```python
from build123d import *

# Parameters (mm, degrees)
SKETCH1_W           = 300
SKETCH1_H           = 80
BOSS_EXTRUDE1_DEPTH = 8
M8_TAPPED_HOLE1_D   = 6.8


with BuildPart() as part:
    # Sketch1 → Boss-Extrude1 (new body)
    with BuildSketch(Plane(origin=(0, 0, 0), x_dir=(1, 0, 0), z_dir=(0, 1, 0))):
        with Locations((150, 40)):
            Rectangle(SKETCH1_W, SKETCH1_H)
    extrude(amount=BOSS_EXTRUDE1_DEPTH)

    # M8 Tapped Hole1 (through all)
    with Locations(Plane(origin=(0, 8, 0), x_dir=(1, 0, 0), z_dir=(0, 1, 0))):
        with Locations((50, 40), (250, 40)):
            Hole(M8_TAPPED_HOLE1_D / 2)


solid = part.part
```
Model file for the job. Use its own axes, mm. Coordinates: 2 decimals unless noted, no trailing zeros. Loops run counter-clockwise (first coordinate to the right, second up) from the corner with the lowest first, then second, coordinate; pieces in that order, holes last. Notation, with made-up numbers: M 48.5,69.5 L 71.5,69.5 A14 ccw 71.5,95.5 Z; hole C 54.25,27.5 d2. An arc over 180 degrees is marked long. Use CSV: the item, a comma, the result in double quotes. Start each with the question number.
1. Probe probe 1 along X at (y, z) = (2, -40); probe 2 along Z at (x, y) = (250, 3.5). List the from-to ranges inside material, lowest first. Write a range as [from, to].
2. Flat gauge pin, fed straight in: pin 1 (3 mm diameter, centred on y = 3.5, z = -53.5, fed in from -X). Where does the tip first touch, or does it go through?
3. Two-plate mould, pull along X, no slides. Class faces 1 (the cylindrical face through (46.86, 3.94, -38.7)), 2 (the flat face through (0, 4, -39)), 3 (the flat face through (148, 4, -80)), 4 (the cylindrical face through (246.757, 3.944, -41.021)): pulls with the +X half, pulls with the -X half, needs draft (parallel to the pull), parting line crosses it, or undercut.
4. Band-saw the part on A-A, the plane z = -40. List the corners of the cut face in (x, y).
5. Band-saw the part on B-B, the plane x = 250. List the corners of the cut face in (y, z), then the cut area to 3 significant figures.
Entries:
1,probe 1,"x = [0, 46.6], [53.4, 246.6], [253.4, 300]"
1,probe 2,"z = [-80, -43.4], [-36.6, 0]"
2,pin 1,"stops at x = 0"
3,face 1,"undercut"
3,face 2,"pulls with the -X half"
3,face 3,"needs draft"
3,face 4,"undercut"
4,outline,"M 0,0 L 46.6,0 L 46.6,8 L 0,8 Z; M 53.4,0 L 246.6,0 L 246.6,8 L 53.4,8 Z; M 253.4,0 L 300,0 L 300,8 L 253.4,8 Z"
5,outline,"M 0,-80 L 8,-80 L 8,-43.4 L 0,-43.4 Z; M 0,-36.6 L 8,-36.6 L 8,0 L 0,0 Z"
5,area,"586 mm2"
